The model under review builds one solid part; all positions refer to its coordinate system, in mm. A direction names the side the tool comes from. Round coordinates to 2 decimals unless told otherwise and drop trailing zeros. Write each loop counter-clockwise with the first axis right and the second up, starting at its lowest first coordinate (ties: lowest second). Pieces come first, ordered by that corner, then holes. Notation, with made-up numbers: (-9, -16.5) -> (46, -16.5) arc R24 ccw to (46, 0.5) -> close; hole circle Ø3 at (39.25, 83.25). An arc over 180 degrees is marked (long way). Use CSV: the item, a comma, the result in double quotes. Start each with the question number.
1) Take a section at A-A, the plane y = 603. Give the boundary of the cut face in (x, z), then the cut area to 3 significant figures.
2) Mouldability with a two-part tool opening along Z and no side actions: class faces 1 (the face through (-450, 350, 13)), 2 (the face through (-450, 364, -11)), 3 (the face through (-427, 350, 0)) as released by +Z, released by -Z, zero draft, split by the parting line, or undercut.
3) Machinability: for faces 4 (the face through (-476, 11, -2.5)), 5 (the face through (-450, 350, -13)), 6 (the face through (-476, 11, 2.5)), 7 (the face through (-450, 364, 11)), 8 (the face through (-424, 11, -2.5)), which of the approach directions +Z, -Z, +X, -X, +Y, -Y give a long, thin tool a straight path to every point of the face, cutting with its end or side? Answer none if there is none.
4) Wall thickness on probe 1 along Z at (x, y) = (-461, 415); probe 2 along X at (y, z) = (589, 9); probe 3 along Y at (x, z) = (-443, -16): over which ranges is each line inside the solid? List them lowest first. Write a range as [from, to].
5) Take a section at B-B, the plane x = -462.5. Give the boundary of the cut face in (y, z), then the cut area to 3 significant figures.
6) For pin 1 Ø1 at (x, y) = (-446, 529) entering from -Z; pin 2 Ø8 at (y, z) = (303, 3.5) entering from -X; pin 3 Ø9.5 at (x, y) = (-420.5, 13.5) entering from -Z; pin 4 Ø4 at (x, z) = (-473, -8) entering from -Y, all flat-tipped, find the tip position at first contact; note any pin that passes through.
from build123d import *

# Parameters (mm, degrees)
SKETCH2_W           = 70
SKETCH2_H           = 50
BOSS_EXTRUDE1_DEPTH = 5
SKETCH3_W           = 46
SKETCH3_H           = 26
BOSS_EXTRUDE2_DEPTH = 700
BOSS_EXTRUDE3_DEPTH = 2.5
SKETCH5_W           = 42
SKETCH5_H           = 22
CUT_EXTRUDE1_DEPTH  = 691


with BuildPart() as part:
    # Sketch2 → Boss-Extrude1 (new body)
    with BuildSketch(Plane(origin=(0, 0, 0), x_dir=(1, 0, 0), z_dir=(0, 1, 0))):
        with Locations((-450, 0)):
            Rectangle(SKETCH2_W, SKETCH2_H)
    extrude(amount=BOSS_EXTRUDE1_DEPTH)

    # Sketch3 → Boss-Extrude2 (add)
    with BuildSketch(Plane(origin=(0, 5, 0), x_dir=(1, 0, 0), z_dir=(0, 1, 0))):
        with Locations((-450, 0)):
            Rectangle(SKETCH3_W, SKETCH3_H)
    extrude(amount=BOSS_EXTRUDE2_DEPTH)

    # Sketch4 → Boss-Extrude3 (add, symmetric)
    with BuildSketch(Plane.XY):
        Polygon((-473, 5), (-485, 5), (-473, 25), align=None)
        Polygon((-427, 25), (-427, 5), (-415, 5), align=None)
    extrude(amount=BOSS_EXTRUDE3_DEPTH, both=True)

    # Sketch5 → Cut-Extrude1 (cut)
    with BuildSketch(Plane(origin=(0, 705, 0), x_dir=(1, 0, 0), z_dir=(0, 1, 0))):
        with Locations((-450, 0)):
            Rectangle(SKETCH5_W, SKETCH5_H)
    extrude(amount=-CUT_EXTRUDE1_DEPTH, mode=Mode.SUBTRACT)


solid = part.part
Values found:
1,outline,"(-473, -13) -> (-427, -13) -> (-427, 13) -> (-473, 13) -> close; hole (-471, -11) -> (-429, -11) -> (-429, 11) -> (-471, 11) -> close"
1,area,"272 mm²"
2,face 1,"released by +Z"
2,face 2,"undercut"
2,face 3,"zero draft"
3,face 4,"-Z, -X, +Y"
3,face 5,"-Z, +X, -X, +Y"
3,face 6,"+Z, -X, +Y"
3,face 7,"+Y"
3,face 8,"-Z, +X, +Y"
4,probe 1,"[-13, -11], [11, 13]"
4,probe 2,"[-473, -471], [-429, -427]"
4,probe 3,"[0, 5]"
5,outline,"(0, -25) -> (5, -25) -> (5, -13) -> (705, -13) -> (705, -11) -> (14, -11) -> (14, 11) -> (705, 11) -> (705, 13) -> (5, 13) -> (5, 25) -> (0, 25) -> close"
5,area,"3,250 mm²"
6,pin 1,"z = -13"
6,pin 2,"x = -473"
6,pin 3,"z = -2.5"
6,pin 4,"y = 0"
